from build123d import *

# Parameters (mm, degrees)
SKETCH1_W           = 40
SKETCH1_H           = 80
SKETCH1_R           = 12
BOSS_EXTRUDE1_DEPTH = 14


with BuildPart() as part:
    # Sketch1 → Boss-Extrude1 (new body)
    with BuildSketch(Plane.XY):
        with Locations((20, 40)):
            Rectangle(SKETCH1_W, SKETCH1_H)
        with Locations((20, 40)):
            Circle(SKETCH1_R, mode=Mode.SUBTRACT)
    extrude(amount=BOSS_EXTRUDE1_DEPTH)


solid = part.part
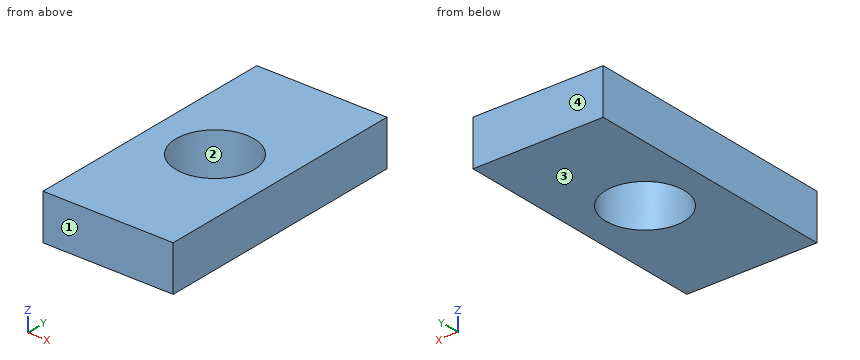
CAD build for the part. Positions are in the model's coordinates, mm. Face numbers are marked on the shaded views. Round coordinates to 2 decimals unless told otherwise and drop trailing zeros. Write each loop counter-clockwise with the first axis right and the second up, starting at its lowest first coordinate (ties: lowest second). Pieces come first, ordered by that corner, then holes.
(1) Slice it at A-A, the plane x = 20. Write the cut outline in (y, z).
(2) Slice it at C-C, the plane y = 40. Write the cut outline in (x, z).
(3) Slice it at B-B, the plane z = 5. Write the cut outline in (x, y), and give its area (3 significant figures).
(4) Probe line 1 along Y through (x, z) = (20, 9); line 2 along X through (y, z) = (40.5, 6); line 3 along X through (y, z) = (47.5, 9). List the from-to ranges inside material, lowest first.
(5) Mould opens along Y. For the marked faces 1, 2, 3 and 4 say: pulls with the +Y half, pulls with the -Y half, needs draft (parallel to the pull), parting line crosses it, or undercut.
From the geometry:
1. outline: (0, 0) - (28, 0) - (28, 14) - (0, 14) - close; (52, 0) - (80, 0) - (80, 14) - (52, 14) - close
2. outline: (0, 0) - (8, 0) - (8, 14) - (0, 14) - close; (32, 0) - (40, 0) - (40, 14) - (32, 14) - close
3. outline: (0, 0) - (40, 0) - (40, 80) - (0, 80) - close; hole circle Ø24 at (20, 40)
3. area: 2,750 mm2
4. line 1: y = 0 to 28, 52 to 80
4. line 2: x = 0 to 8.01, 31.99 to 40
4. line 3: x = 0 to 10.63, 29.37 to 40
5. face 1: pulls with the -Y half
5. face 2: undercut
5. face 3: needs draft
5. face 4: pulls with the +Y half
